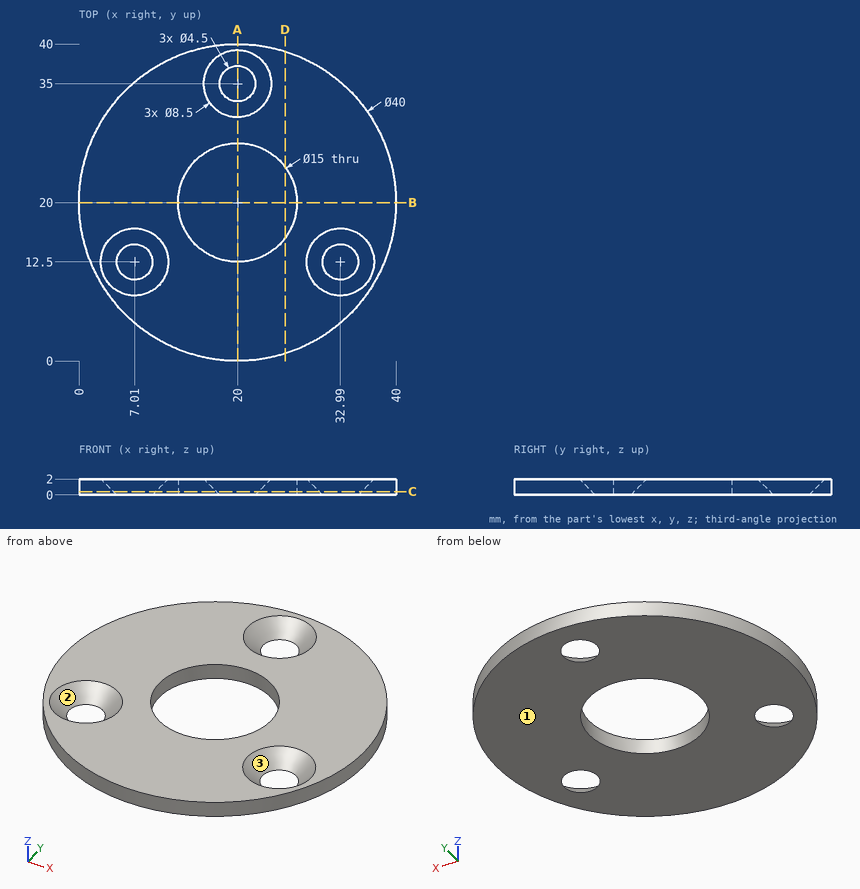
Source: three-view drawing plus pictorial views. Frame: mm from the lowest corner of the part. Give positions to 0.01 mm unless a question says otherwise; leave off trailing zeros. Write each loop counter-clockwise with the first axis right and the second up, starting at its lowest first coordinate (ties: lowest second). Pieces come first, ordered by that corner, then holes. Notation, with made-up numbers: M 41,27.5 L 64,27.5 A13 ccw 64,45.5 Z; hole C 89.25,69.25 d10. An arc over 180 degrees is marked long. Use one line per item in the form item = value.
1. Cut plane A-A on x = 20. Return loops of the section in (y, z).
Outcome:
outline = M 0,0 L 12.5,0 L 12.5,2 L 0,2 Z; M 27.5,0 L 32.75,0 L 30.75,2 L 27.5,2 Z; M 37.25,0 L 40,0 L 40,2 L 39.25,2 Z
2. Cut plane B-B on y = 20. Return loops of the section in (x, z).
Outcome:
outline = M 0,0 L 12.5,0 L 12.5,2 L 0,2 Z; M 27.5,0 L 40,0 L 40,2 L 27.5,2 Z
3. Cut plane C-C on z = 0.4. State how many separate pieces and enclosed holes the cut face has, and give its area (3 significant figures).
Outcome:
separate_pieces = 1
enclosed_holes = 4
area = 1,010 mm²
4. Ray query, L1, parallel to Y at x = 20, z = 1.3; L2, parallel to Y at x = 20, z = 0.4; L3, parallel to Y at x = 24, z = 1.3 (1 decimal). Return the intervals inside material, ascending.
Outcome:
L1 = 0 to 12.5, 27.5 to 31.45, 38.55 to 40
L2 = 0 to 12.5, 27.5 to 32.35, 37.65 to 40
L3 = 0.4 to 13.7, 26.3 to 39.6
5. Mould query, pull axis X, two halves, no side actions, for the marked faces 1, 2 and 3. Classes: released by +X, released by -X, zero draft, split by the parting line, or undercut.
Outcome:
face_1 = zero draft
face_2 = undercut
face_3 = undercut
6. Cut plane D-D on x = 26. Return loops of the section in (y, z).
Outcome:
outline = M 0.92,0 L 15.5,0 L 15.5,2 L 0.92,2 Z; M 24.5,0 L 39.08,0 L 39.08,2 L 24.5,2 Z
